The model under review builds one solid part; all positions refer to its coordinate system, in mm. A direction names the side the tool comes from. Coordinates: 2 decimals unless noted, no trailing zeros. Order: outer loops, then holes, each group sorted by start corner. A loop starts at its lowest first (then second) coordinate and runs counter-clockwise, first axis right, second up. Notation, with made-up numbers: M -37,51 L -7,51 A23 cw -7,69 Z; hole C 39.25,-39.5 d10. An arc over 180 degrees is marked long. Answer in a Markdown table with one row per item.
from build123d import *

# Parameters (mm, degrees)
EXTRUDE_THIN1_DEPTH = 1062


with BuildPart() as part:
    # Sketch1 → Extrude-Thin1 (new, symmetric)
    with BuildSketch(Plane(origin=(0, 0, 0), x_dir=(1, 0, 0), z_dir=(0, 1, 0))):
        with BuildLine():
            Line((-50, 30), (50, 30))
            ThreePointArc((50, 30), (57.071067812, 27.071067812), (60, 20))
            Line((60, 20), (60, -20))
            ThreePointArc((60, -20), (57.071067812, -27.071067812), (50, -30))
            Line((50, -30), (-50, -30))
            ThreePointArc((-50, -30), (-57.071067812, -27.071067812), (-60, -20))
            Line((-60, -20), (-60, 20))
            ThreePointArc((-60, 20), (-57.071067812, 27.071067812), (-50, 30))
        make_face()
        with BuildLine():
            Line((-50, 26), (50, 26))
            ThreePointArc((50, 26), (54.242640687, 24.242640687), (56, 20))
            Line((56, 20), (56, -20))
            ThreePointArc((56, -20), (54.242640687, -24.242640687), (50, -26))
            Line((50, -26), (-50, -26))
            ThreePointArc((-50, -26), (-54.242640687, -24.242640687), (-56, -20))
            Line((-56, -20), (-56, 20))
            ThreePointArc((-56, 20), (-54.242640687, 24.242640687), (-50, 26))
        make_face(mode=Mode.SUBTRACT)
    extrude(amount=EXTRUDE_THIN1_DEPTH, both=True)


solid = part.part
(1) Take a section at C-C (z = -0.5). Write out the cut boundary in (x, y).
Report:
| item | result |
|---|---|
| outline | M -60,-1062 L -56,-1062 L -56,1062 L -60,1062 Z; M 56,-1062 L 60,-1062 L 60,1062 L 56,1062 Z |
(2) Insertion check: P1, Ø1, axis at y = -253, z = -21, coming from the +X side. The pin has a flat end and moves straight along its axis. Give the tip position at first contact, or say it passes through.
Report:
| item | result |
|---|---|
| P1 | x = 59.99 |
(3) The part is to be moulded in two halves that separate along Z. For faces 1 (the flat face through (-56, 15, 0)), 2 (the flat face through (-60, 15, 0)), 3 (the flat face through (-1, 15, -30)), say which applies: +Z half, -Z half, draft (parallel to the pull), parting line (faces both ways), or undercut.
Report:
| item | result |
|---|---|
| face 1 | undercut |
| face 2 | draft |
| face 3 | -Z half |
(4) Take a section at A-A (x = -31). Write out the cut boundary in (y, z).
Report:
| item | result |
|---|---|
| outline | M -1062,-30 L 1062,-30 L 1062,-26 L -1062,-26 Z; M -1062,26 L 1062,26 L 1062,30 L -1062,30 Z |
(5) Machinability: for faces 4 (the flat face through (1, 15, 30)), 5 (the flat face through (-1, 15, -26)), which of the approach directions +Z, -Z, +X, -X, +Y, -Y give a long, thin tool a straight path to every point of the face, cutting with its end or side? Answer none if there is none.
Report:
| item | result |
|---|---|
| face 4 | +Z, +X, -X, +Y, -Y |
| face 5 | +Y, -Y |
(6) Take a section at B-B (y = -933). Write out the cut boundary in (x, z), then the cut area to 3 significant figures.
Report:
| item | result |
|---|---|
| outline | M -60,-20 A10 ccw -50,-30 L 50,-30 A10 ccw 60,-20 L 60,20 A10 ccw 50,30 L -50,30 A10 ccw -60,20 Z; hole M -56,-20 A6 ccw -50,-26 L 50,-26 A6 ccw 56,-20 L 56,20 A6 ccw 50,26 L -50,26 A6 ccw -56,20 Z |
| area | 1,320 mm^2 |
(7) To check wall thickness, follow line 1 (X direction, y = -381.5, z = -4); line 2 (Z direction, x = 25, y = 821); line 3 (X direction, y = -304, z = 21.5). State the ranges of each line that lie inside material, in increasing order. Write a range as [from, to].
Report:
| item | result |
|---|---|
| line 1 | [-60, -56], [56, 60] |
| line 2 | [-30, -26], [26, 30] |
| line 3 | [-59.89, -55.81], [55.81, 59.89] |
